Design review of the part built by this model. Coordinates are the model's own, in mm. A direction names the side the tool comes from. Coordinates: 2 decimals unless noted, no trailing zeros. Loops run counter-clockwise (first coordinate to the right, second up) from the corner with the lowest first, then second, coordinate; pieces in that order, holes last. Notation, with made-up numbers: M -9,-11.75 L 40,-11.75 A8 ccw 40,-0.75 Z; hole C 19.5,3.5 d8. An arc over 180 degrees is marked long. Write item = value, one per line. Start each with the question number.
from build123d import *

# Parameters (mm, degrees)
BASE_START          = -20
BASE_FLAT_DEPTH     = 20
CROSS_HOLE_SKETCH_R = 4
CROSS_HOLE_8_DEPTH  = 30
EDGE_FILLET_R2_R    = 2
SLOT_2X16_DEPTH     = 2


with BuildPart() as part:
    # Shaft Profile Sketch → Stepped Shaft Body (revolve)
    with BuildSketch(Plane.XY, mode=Mode.PRIVATE) as stepped_shaft_body_sk:
        Polygon((4, 72), (4, 0), (18, 0), (18, 24), (14, 24), (14, 48), (10, 48), (10, 72), align=None)
    revolve(stepped_shaft_body_sk.sketch.rotate(Axis((0, -40.631578947, 0), (0, 1, 0)), 90), axis=Axis((0, -40.631578947, 0), (0, 1, 0)))

    # Base Flat Sketch → Base Flat (cut)
    with BuildSketch(Plane.XZ.offset(BASE_START)):
        with BuildLine():
            Line((-14, 11.313708499), (-14, -11.313708499))
            ThreePointArc((-14, -11.313708499), (-18, 0), (-14, 11.313708499))
        make_face()
        with BuildLine():
            Line((14, 11.313708499), (14, -11.313708499))
            ThreePointArc((14, -11.313708499), (18, 0), (14, 11.313708499))
        make_face()
    extrude(amount=BASE_FLAT_DEPTH, mode=Mode.SUBTRACT)

    # Cross Hole Sketch → Cross Hole Ø8 (cut)
    with BuildSketch(Plane.ZY.offset(14)):
        with Locations((0, 10)):
            Circle(CROSS_HOLE_SKETCH_R)
    extrude(amount=-CROSS_HOLE_8_DEPTH, mode=Mode.SUBTRACT)

    # Edge Fillet R2
    edge_fillet_r2_edges = [part.edges().sort_by_distance(p)[0] for p in [
        (0, 72, 10),
    ]]
    fillet(edge_fillet_r2_edges, radius=EDGE_FILLET_R2_R)

    # Slot Sketch → Slot 2x16 (cut)
    with BuildSketch(Plane(origin=(8, 0, 0), x_dir=(0, 0, -1), z_dir=(1, 0, 0))):
        with BuildLine():
            Line((2, 65.548124709), (2, 53.548124709))
            ThreePointArc((2, 53.548124709), (0, 51.548124709), (-2, 53.548124709))
            Line((-2, 53.548124709), (-2, 65.548124709))
            ThreePointArc((-2, 65.548124709), (0, 67.548124709), (2, 65.548124709))
        make_face()
    slot_2x16 = extrude(amount=SLOT_2X16_DEPTH, mode=Mode.SUBTRACT)

    # Slot Mirror: Slot 2x16 across plane
    add(slot_2x16.mirror(Plane(origin=(0, 0, 0), x_dir=(0, 0, 1), z_dir=(1, 0, 0))), mode=Mode.SUBTRACT)


solid = part.part
Q1. Add section B-B on x = 11.5. State the section outline as (y, z) points, plus the area to 3 significant figures.
Q2. For faces 4 (the face through (14, 15, 0)), 5 (the face through (-8, 60, 0)), 6 (the face through (11, 24, -9)), 7 (the face through (9, 59, 2)), 8 (the face through (8.458, 8.468, 3.695)), list the 3-axis set-ups (+Z, -Z, +X, -X, +Y, -Y) from which the entire face can be reached by the end or side of a thin tool; tool diameter is ignored.
Q3. To check wall thickness, follow line 1 (Y direction, x = 8.5, z = 0); line 2 (X direction, y = 3, z = 0); line 3 (Y direction, x = 9, z = -1). State the ranges of each line that lie inside material, in increasing order. Write a range as from..to.
Q4. Mouldability with a two-part tool opening along Z and no side actions: class faces 1 (the face through (-9, 60, -2)), 2 (the face through (-16, 20, 0)), 3 (the face through (-0.791, 14.835, 17.983)) as released by +Z, released by -Z, zero draft, split by the parting line, or undercut.
Q5. Add section A-A on z = 0. Give the number of separate pieces and of enclosed holes in the cut face, plus the area to 3 significant figures.
Q6. Clearance check with flat-ended pins moving along their axes: P1, Ø0.9, axis at x = 8.5, y = 57, coming from the +Z side; P2, Ø12, axis at y = 27.5, z = -10, coming from the +X side; P3, Ø8, axis at x = 0, z = -7, coming from the -Y side; P4, Ø5, axis at x = 0, y = 59, coming from the +Z side. State where each tip first meets the part, or that it passes through.
Values follow:
q1.outline = M 0,-13.85 L 24,-13.85 L 24,-7.98 L 48,-7.98 L 48,7.98 L 24,7.98 L 24,13.85 L 0,13.85 Z; hole C 10,0 d8
q1.area = 998 mm2
q2.face_4 = +Z, -Z, +X, -Y
q2.face_5 = -X
q2.face_6 = +Y
q2.face_7 = +X
q2.face_8 = +X, -X
q3.line_1 = 0..6, 14..51.55, 67.55..71.94
q3.line_2 = -14..-4, 4..14
q3.line_3 = 0..6.13, 13.87..51.82, 67.28..71.7
q4.face_1 = undercut
q4.face_2 = zero draft
q4.face_3 = split by the parting line
q5.separate_pieces = 4
q5.enclosed_holes = 0
q5.area = 1,050 mm2
q6.P1 = 5.93
q6.P2 = 17.25
q6.P3 = 0
q6.P4 = 10
